Build history of the part. All positions in model axes, mm. Round coordinates to 2 decimals unless told otherwise and drop trailing zeros. One line per question, with ' | ' between items.
from build123d import *

# Parameters (mm, degrees)
SKETCH_1_W                   = 200
SKETCH_1_H                   = 570
EXTRUDE_1_DEPTH              = 15
CHAMFER_1_SIZE               = 5
MM_0_D                       = 6
HOLE_WIZARD_M6_1_D           = 5
HOLE_WIZARD_M5_2_D           = 4.2
HOLE_WIZARD_M6_2_D           = 5
HOLE_WIZARD_M4_1_D           = 3.3
MM_1_D                       = 1
MM_1_DEPTH                   = 17
MM_1_TIP                     = 0.30043031
HOLE_WIZARD_M5_1_D           = 5.5
HOLE_WIZARD_M5_1_DEPTH       = 17
HOLE_WIZARD_M5_1_CBORE_D     = 10
HOLE_WIZARD_M5_1_CBORE_DEPTH = 7
HOLE_WIZARD_M5_1_TIP         = 1.652366702
HOLE_WIZARD_1_D              = 6.6
HOLE_WIZARD_1_CBORE_D        = 11
HOLE_WIZARD_1_CBORE_DEPTH    = 7


with BuildPart() as part:
    # 草图1 → 凸台-拉伸1 (new body)
    with BuildSketch(Plane.XY):
        Rectangle(SKETCH_1_W, SKETCH_1_H)
    extrude(amount=EXTRUDE_1_DEPTH)

    # 倒角1
    chamfer_1_edges = [part.edges().sort_by_distance(p)[0] for p in [
        (100, -285, 7.5),
        (-100, -285, 7.5),
        (-100, 285, 7.5),
        (100, 285, 7.5),
    ]]
    chamfer(chamfer_1_edges, length=CHAMFER_1_SIZE)

    # 大小mm 暗销孔0 (through all)
    with Locations(Plane.XY.offset(15)):
        with Locations((-42, -193), (258, -193), (-42, 193), (258, 193)):
            Hole(MM_0_D / 2)

    # M6 螺纹孔1 (through all)
    with Locations(Plane.XY.offset(15)):
        with Locations((55, 196), (25, 196), (55, -196), (25, -196)):
            Hole(HOLE_WIZARD_M6_1_D / 2)

    # M5 螺纹孔2 (through all)
    with Locations(Plane.XY.offset(15)):
        with Locations((-55, 240), (-55, 180), (-55, 120), (-55, 60), (-55, 0), (-55, -60), (-55, -120), (-55, -180)):
            Hole(HOLE_WIZARD_M5_2_D / 2)

    # M6 螺纹孔2 (through all)
    with Locations(Plane.XY.offset(15)):
        with Locations((-92.500000001, -277.499999995), (-17.500000001, -277.499999995), (-17.499999995, 277.500000015), (-92.499999995, 277.500000015)):
            Hole(HOLE_WIZARD_M6_2_D / 2)

    # M4 螺纹孔1 (through all)
    with Locations(Plane.XY.offset(15)):
        with Locations((90, -160), (90, -90), (90, 90), (90, 160)):
            Hole(HOLE_WIZARD_M4_1_D / 2)

    # 大小mm 暗销孔1
    with Locations(Plane(origin=(0, 0, 0), x_dir=(-1, 0, 0), z_dir=(0, 0, -1))):
        with Locations((24.5, 103), (-75.5, 103), (24.5, -147), (-75.5, -147), (24.5, 3), (-75.5, 3)):
            Hole(MM_1_D / 2, depth=MM_1_DEPTH)
            with Locations((0, 0, -(MM_1_DEPTH + MM_1_TIP / 2))):  # 118° drill point
                Cone(0, MM_1_D / 2, MM_1_TIP, mode=Mode.SUBTRACT)

    # M5 六角凹头螺钉的柱形沉头孔1
    with Locations(Plane.XY.offset(15)):
        with Locations((75.5, -147), (75.5, 103), (75.5, 3), (-24.5, 103), (-24.5, 3), (-24.5, -147)):
            CounterBoreHole(HOLE_WIZARD_M5_1_D / 2, HOLE_WIZARD_M5_1_CBORE_D / 2, HOLE_WIZARD_M5_1_CBORE_DEPTH, depth=HOLE_WIZARD_M5_1_DEPTH)
            with Locations((0, 0, -(HOLE_WIZARD_M5_1_DEPTH + HOLE_WIZARD_M5_1_TIP / 2))):  # 118° drill point
                Cone(0, HOLE_WIZARD_M5_1_D / 2, HOLE_WIZARD_M5_1_TIP, mode=Mode.SUBTRACT)

    # 打孔尺寸(%根据)内六角花形圆柱头螺钉1 (through all)
    with Locations(Plane.XY.offset(15)):
        with Locations((-80, -225), (80, -225), (-80, 225), (80, 225)):
            CounterBoreHole(HOLE_WIZARD_1_D / 2, HOLE_WIZARD_1_CBORE_D / 2, HOLE_WIZARD_1_CBORE_DEPTH)


solid = part.part
Q1. Pull direction Y, two halves, no side cores. Call faces 1 (the cylindrical face through (80.119, -148.915, 11.549)), 2 (the flat face through (-1, -285, 7)), 3 (the flat face through (-100, -4, 7)): +Y half, -Y half, draft (parallel to the pull), parting line (faces both ways), or undercut.
Found:
face 1: undercut | face 2: -Y half | face 3: draft
Q2. Drop flat-ended pins along their axis: pin 1 (3.5 mm diameter, centred on x = 77.5, y = -224, fed in from +Z); pin 2 (9 mm diameter, centred on x = 81.5, y = 224, fed in from +Z). Give the stop position or say it passes through.
Found:
pin 1: z = 8 | pin 2: z = 15
Q3. Drill centre lines: L1, parallel to Y at x = -92.5, z = 11.75; L2, parallel to Y at x = -81, z = 8.5; L3, parallel to Y at x = -24.5, z = 1.5. Where is each one in solid material? Low to high. Write a range as from..to.
Found:
L1: -285..-280, -275..275, 280..285 | L2: -285..-230.41, -219.59..219.59, 230.41..285 | L3: -285..-149.75, -144.25..0.25, 5.75..100.25, 105.75..285
